Read the model definition and answer for the solid it produces. Units are mm, in the model's axes. A direction names the side the tool comes from. Coordinates: 2 decimals unless noted, no trailing zeros. Loops run counter-clockwise (first coordinate to the right, second up) from the corner with the lowest first, then second, coordinate; pieces in that order, holes last. Notation, with made-up numbers: M 84,-29 L 88,-29 A29 ccw 88,2 Z; hole C 42.5,8.5 d3. An arc over 180 degrees is marked long. One line per item, written item: value. Start each with the question number.
```python
from build123d import *

# Parameters (mm, degrees)
LINK_PLATE_PROFILE_R      = 8
LINK_PLATE_PROFILE_R_2    = 13
LINK_PLATE_DEPTH          = 24
HUB_DISC_PROFILE_84_R     = 42
HUB_DISC_84_DEPTH         = 10
HUB_RIB_DEPTH             = 5
HUB_CENTRE_BORE_SKETCH_R  = 13
HUB_CENTRE_BORE_DEPTH     = 127.791166885
HUB_HOLE_SKETCH_R         = 5
HUB_HOLE_DEPTH            = 127.791166885
HUB_HOLE_PATTERN_8X_COUNT = 8


with BuildPart() as part:
    # Link Plate Profile → Link Plate (new body)
    with BuildSketch(Plane.XY):
        with BuildLine():
            ThreePointArc((-65.704893873, -50.938461538), (-46.286814024, -0.688477763), (-56.99168633, 52.108571429))
            ThreePointArc((-56.99168633, 52.108571429), (-94.004081038, 61.906293942), (-100.648486627, 24.2))
            ThreePointArc((-100.648486627, 24.2), (-90.130360042, -3.018741212), (-95.928832541, -31.617142857))
            ThreePointArc((-95.928832541, -31.617142857), (-89.695133026, -55.165895806), (-65.704893873, -50.938461538))
        make_face()
        with Locations((-80, -40)):
            Circle(LINK_PLATE_PROFILE_R, mode=Mode.SUBTRACT)
        with BuildLine():
            ThreePointArc((-81.86521747, 7.908967037), (-81.11107364, 12.018176986), (-77.500675884, 14.120406128))
            ThreePointArc((-77.500675884, 14.120406128), (-70.565087966, 15.772279618), (-64.338947731, 19.245929512))
            ThreePointArc((-64.338947731, 19.245929512), (-59.317592319, 19.833129635), (-56.350771542, 15.739623969))
            ThreePointArc((-56.350771542, 15.739623969), (-56.717251337, -4.095758702), (-61.619133807, -23.319396791))
            ThreePointArc((-61.619133807, -23.319396791), (-64.890999648, -26.333889771), (-69.26986273, -25.547866796))
            ThreePointArc((-69.26986273, -25.547866796), (-72.768447006, -23.516534306), (-76.632322996, -22.317840867))
            ThreePointArc((-76.632322996, -22.317840867), (-79.776843452, -20.296408854), (-80.640782737, -16.659403878))
            ThreePointArc((-80.640782737, -16.659403878), (-80.022314885, -4.313883718), (-81.86521747, 7.908967037))
        make_face(mode=Mode.SUBTRACT)
        with Locations((-80, 40)):
            Circle(LINK_PLATE_PROFILE_R_2, mode=Mode.SUBTRACT)
    extrude(amount=LINK_PLATE_DEPTH)



with BuildPart() as body_2:
    # Hub Disc Profile Ø84 → Hub Disc Ø84 (new, symmetric)
    with BuildSketch(Plane.XY.offset(12)):
        Circle(HUB_DISC_PROFILE_84_R)
    extrude(amount=HUB_DISC_84_DEPTH, both=True)


with BuildPart() as part_1:
    add(part.part)

    add(body_2.part)  # Hub Rib merges body 2
    # Rib Profile → Hub Rib (add, symmetric)
    with BuildSketch(Plane.XY.offset(12)):
        with BuildLine():
            Line((-80, 66), (5.116324571, 41.687206945))
            ThreePointArc((5.116324571, 41.687206945), (-41.921728803, 2.562938577), (0, -42))
            Line((0, -42), (-80, -58))
            ThreePointArc((-80, -58), (-57.293928807, 4), (-80, 66))
        make_face()
    extrude(amount=HUB_RIB_DEPTH, both=True)

    # Hub Centre Bore Sketch → Hub Centre Bore (cut, through all)
    with BuildSketch(Plane.XY.offset(22)):
        Circle(HUB_CENTRE_BORE_SKETCH_R)
    extrude(amount=-HUB_CENTRE_BORE_DEPTH, mode=Mode.SUBTRACT)

    # Hub Hole Sketch → Hub Hole (cut, through all)
    with BuildSketch(Plane.XY.offset(22)):
        with Locations((0, 30)):
            Circle(HUB_HOLE_SKETCH_R)
    hub_hole = extrude(amount=-HUB_HOLE_DEPTH, mode=Mode.SUBTRACT)

    # Hub Hole Pattern 8x: Hub Hole ×8 about axis
    hub_hole_pattern_8x_axis = Axis((0, 0, 0), (0, 0, 1))
    for i in range(1, HUB_HOLE_PATTERN_8X_COUNT):
        add(hub_hole.rotate(hub_hole_pattern_8x_axis, i * 360 / HUB_HOLE_PATTERN_8X_COUNT), mode=Mode.SUBTRACT)


solid = part_1.part
```
1) For a pull along X with two mould halves and no side action, classify faces 6 (the face through (-36, -49.2, 12.1)), 7 (the face through (-56.68, -3.82, 6.5)), 8 (the face through (-90.01, -54.96, 11.83)), 9 (the face through (25.12, 1.08, 12.14)) as released by +X, released by -X, zero draft, split by the parting line, or undercut.
2) Section B-B (y = 10) is taken. Determine the outline of the cut face in (x, z), then the cut area to 3 significant figures.
3) Section A-A (x = -30) is taken. Determine the outline of the cut face in (y, z), then the cut area to 3 significant figures.
4) Flat-ended cylindrical pins translate along their axes: pin 1 (23.5 mm diameter, centred on x = -15, y = 20.5, fed in from -Z); pin 2 (3.5 mm diameter, centred on x = -58, y = 4.5, fed in from -Z); pin 3 (8 mm diameter, centred on x = 0, y = 30, fed in from +Z); pin 4 (1 mm diameter, centred on x = -71.5, z = 4, fed in from +Y). Find the tip coordinate at first contact, or state that the pin passes through.
5) Section D-D (y = 40) is taken. Determine the outline of the cut face in (x, z), then the cut area to 3 significant figures.
6) Section C-C (x = 23) is taken. Determine the outline of the cut face in (y, z).
7) Consider line 1 along X through (y, z) = (-6, 19); line 2 along X through (y, z) = (-22, 2.25); line 3 along Y through (x, z) = (-17.5, 21.5). Determine where each line is inside the solid, lowest interval first.
8) A tool of negligible diameter and unlimited length cuts with its end or side. For faces 1 (the face through (-57.38, -0.09, 12.07)), 2 (the face through (40.06, 12.62, 12.14)), 3 (the face through (9, 10, 22)), 4 (the face through (-83, 5, 0)), 5 (the face through (-42.5, 3, 17)), from which of +Z, -Z, +X, -X, +Y, -Y can it reach the whole face along a straight path? Write none if from no direction.
Results found:
1. face 6: released by +X
1. face 7: undercut
1. face 8: split by the parting line
1. face 9: undercut
2. outline: M -92.94,0 L -81.95,0 L -81.95,24 L -92.94,24 Z; M -57.48,7 L -55.98,7 L -55.98,0 L -45.98,0 L -45.98,7 L -40.79,7 L -40.79,2 L -8.31,2 L -8.31,22 L -40.79,22 L -40.79,17 L -45.98,17 L -45.98,24 L -55.98,24 L -55.98,17 L -57.48,17 Z; M 8.31,2 L 40.79,2 L 40.79,22 L 8.31,22 Z
2. area: 1,870 mm²
3. outline: M -48,7 L -29.39,7 L -29.39,2 L -5,2 L -5,22 L -29.39,22 L -29.39,17 L -48,17 Z; M 5,2 L 29.39,2 L 29.39,7 L 51.72,7 L 51.72,17 L 29.39,17 L 29.39,22 L 5,22 Z
3. area: 1,390 mm²
4. pin 1: stops at z = 2
4. pin 2: stops at z = 7
4. pin 3: passes through
4. pin 4: stops at y = 64.74
5. outline: M -106,0 L -93,0 L -93,24 L -106,24 Z; M -67,0 L -51.65,0 L -51.65,7 L -12.81,7 L -12.81,2 L 12.81,2 L 12.81,22 L -12.81,22 L -12.81,17 L -51.65,17 L -51.65,24 L -67,24 Z
5. area: 1,580 mm²
6. outline: M -35.14,2 L -25.88,2 L -25.88,22 L -35.14,22 Z; M -16.54,2 L 16.54,2 L 16.54,22 L -16.54,22 Z; M 25.88,2 L 35.14,2 L 35.14,22 L 25.88,22 Z
7. line 1: x = -89.96 to -79.96, -57 to -46.89, -41.57 to -11.53, 11.53 to 41.57
7. line 2: x = -92.04 to -77.67, -61.13 to -50.56, -35.78 to -26.15, -16.28 to 16.28, 26.15 to 35.78
7. line 3: y = -38.18 to -24.56, -17.86 to 17.86, 24.56 to 38.18
8. face 1: +Z, -Z
8. face 2: none
8. face 3: +Z, +X, +Y, -Y
8. face 4: -Z, +X, -X, +Y, -Y
8. face 5: +Z
